For this review, take the finished solid that the model builds, in its own axes (mm). A direction names the side the tool comes from. Coordinates: 2 decimals unless noted, no trailing zeros. Order: outer loops, then holes, each group sorted by start corner. A loop starts at its lowest first (then second) coordinate and runs counter-clockwise, first axis right, second up.
from build123d import *

# Parameters (mm, degrees)
SKETCH_1_W                  = 105
SKETCH_1_H                  = 40
EXTRUDE_1_DEPTH             = 18
SKETCH_2_W                  = 30
SKETCH_2_H                  = 40
CUT_EXTRUDE_1_DEPTH         = 5
SKETCH_3_W                  = 60
SKETCH_3_H                  = 40
CUT_EXTRUDE_2_DEPTH         = 6.5
HOLE_WIZARD_1_D             = 6.6
HOLE_WIZARD_1_CBORE_D       = 11
HOLE_WIZARD_1_CBORE_DEPTH   = 6.8
SKETCH_6_R                  = 5
CUT_EXTRUDE_3_DEPTH         = 2
SKETCH_7_R                  = 14
CUT_EXTRUDE_4_DEPTH         = 8
SKETCH_8_R                  = 12.5
CUT_EXTRUDE_5_DEPTH         = 59.021547722
CHAMFER_1_SIZE              = 3
HOLE_WIZARD_M5_1_AT_2_COUNT = 2
HOLE_WIZARD_M5_1_AT_2_PITCH = 10


with BuildPart() as part:
    # 草图1 → 凸台-拉伸1 (new body)
    with BuildSketch(Plane.XY):
        Rectangle(SKETCH_1_W, SKETCH_1_H)
    extrude(amount=EXTRUDE_1_DEPTH)

    # 草图2 → 切除-拉伸1 (cut)
    with BuildSketch(Plane(origin=(0, 0, 0), x_dir=(-1, 0, 0), z_dir=(0, 0, -1))):
        with Locations((37.5, 0)):
            Rectangle(SKETCH_2_W, SKETCH_2_H)
    extrude(amount=-CUT_EXTRUDE_1_DEPTH, mode=Mode.SUBTRACT)

    # 草图3 → 切除-拉伸2 (cut)
    with BuildSketch(Plane(origin=(0, 0, 0), x_dir=(-1, 0, 0), z_dir=(0, 0, -1))):
        with Locations((-22.5, 0)):
            Rectangle(SKETCH_3_W, SKETCH_3_H)
    extrude(amount=-CUT_EXTRUDE_2_DEPTH, mode=Mode.SUBTRACT)

    # 打孔尺寸(%根据)内六角圆柱头螺钉的类型1 (through all)
    with Locations(Plane.XY.offset(18)):
        with Locations((-46, 0), (-30.5, 0), (-15, 0)):
            CounterBoreHole(HOLE_WIZARD_1_D / 2, HOLE_WIZARD_1_CBORE_D / 2, HOLE_WIZARD_1_CBORE_DEPTH)

    # 草图6 → 切除-拉伸3 (cut)
    with BuildSketch(Plane(origin=(0, 0, 0), x_dir=(-1, 0, 0), z_dir=(0, 0, -1))):
        with Locations((15, 0)):
            Circle(SKETCH_6_R)
    extrude(amount=-CUT_EXTRUDE_3_DEPTH, mode=Mode.SUBTRACT)

    # 草图7 → 切除-拉伸4 (cut)
    with BuildSketch(Plane(origin=(0, 0, 6.5), x_dir=(-1, 0, 0), z_dir=(0, 0, -1))):
        with Locations((-17.5, 0)):
            Circle(SKETCH_7_R)
    extrude(amount=-CUT_EXTRUDE_4_DEPTH, mode=Mode.SUBTRACT)

    # 草图8 → 切除-拉伸5 (cut, through all)
    with BuildSketch(Plane(origin=(0, 0, 14.5), x_dir=(-1, 0, 0), z_dir=(0, 0, -1))):
        with Locations((-17.5, 0)):
            Circle(SKETCH_8_R)
    extrude(amount=-CUT_EXTRUDE_5_DEPTH, mode=Mode.SUBTRACT)

    # 倒角1
    chamfer_1_edges = [part.edges().sort_by_distance(p)[0] for p in [
        (-22.5, -20, 2.5),
        (-22.5, 20, 2.5),
        (-7.5, 20, 3.25),
        (-7.5, -20, 3.25),
        (52.5, -20, 12.25),
        (-52.5, -20, 11.5),
        (-52.5, 20, 11.5),
        (52.5, 20, 12.25),
    ]]
    chamfer(chamfer_1_edges, length=CHAMFER_1_SIZE)

    # 草图10 → M5 螺纹孔1 (revolve, cut)
    with BuildSketch(Plane(origin=(44.5, -20, 12.5), x_dir=(0, 0, -1), z_dir=(1, 0, 0))):
        Polygon((0, 0), (0, 13.6618073), (2.1, 12.4), (2.1, 0), align=None)
    hole_wizard_m5_1 = revolve(axis=Axis((44.5, -26.35, 12.5), (0, 1, 0)), mode=Mode.SUBTRACT)

    # M5 螺纹孔1 at 2: M5 螺纹孔1 ×2
    with Locations(*[(-i * HOLE_WIZARD_M5_1_AT_2_PITCH, 0, 0) for i in range(1, HOLE_WIZARD_M5_1_AT_2_COUNT)]):
        add(hole_wizard_m5_1, mode=Mode.SUBTRACT)

    # 镜向1: M5 螺纹孔1 across plane
    add(hole_wizard_m5_1.mirror(Plane.ZX), mode=Mode.SUBTRACT)

    # 镜向1 copy 1 sketch → 镜向1 copy 1 (revolve, cut)
    with BuildSketch(Plane(origin=(34.5, 20, 12.5), x_dir=(0, 0, -1), z_dir=(1, 0, 0))):
        Polygon((0, 0), (0, -13.6618073), (2.1, -12.4), (2.1, 0), align=None)
    revolve(axis=Axis((34.5, 26.35, 12.5), (0, 1, 0)), mode=Mode.SUBTRACT)


solid = part.part
1. Machinability: for faces 5 (the face through (-21, 18.5, 2.5)), 6 (the face through (-7.5, 0, 3)), 7 (the face through (44.39, -6.56, 12.15)), 8 (the face through (-36, 0, 15)), 9 (the face through (22.8, 11.5, 14.5)), which of the approach directions +Z, -Z, +X, -X, +Y, -Y give a long, thin tool a straight path to every point of the face, cutting with its end or side? Answer none if there is none.
Answer below:
face 5: -Z, -X, +Y
face 6: -Z, +X, +Y, -Y
face 7: -Y
face 8: +Z
face 9: -Z
2. The part is to be moulded in two halves that separate along Y. For faces 1 (the face through (51, 18.5, 12.2)), 2 (the face through (-51.495, 0.242, 14.648)), 3 (the face through (-15, -4, 11.2)), 4 (the face through (52.5, 0, 12)), say which applies: +Y half, -Y half, draft (parallel to the pull), parting line (faces both ways), or undercut.
Answer below:
face 1: +Y half
face 2: undercut
face 3: undercut
face 4: draft
3. Take a section at D-D, the plane y = 16. Give the boundary of the cut face in (x, z).
Answer below:
outline: (-52.5, 5) - (-22.5, 5) - (-22.5, 0) - (-7.5, 0) - (-7.5, 6.5) - (52.5, 6.5) - (52.5, 18) - (-52.5, 18) - close; hole circle Ø4.2 at (34.5, 12.5); hole circle Ø4.2 at (44.5, 12.5)
4. Take a section at C-C, the plane y = -10.5. Give the boundary of the cut face in (x, z).
Answer below:
outline: (-52.5, 5) - (-22.5, 5) - (-22.5, 0) - (-7.5, 0) - (-7.5, 6.5) - (8.24, 6.5) - (8.24, 14.5) - (10.72, 14.5) - (10.72, 18) - (-52.5, 18) - close; (24.28, 14.5) - (26.76, 14.5) - (26.76, 6.5) - (52.5, 6.5) - (52.5, 18) - (24.28, 18) - close; hole circle Ø4.2 at (34.5, 12.5); hole circle Ø4.2 at (44.5, 12.5)
5. Take a section at B-B, the plane z = 8. Give the boundary of the cut face in (x, y), plus the area to 3 significant figures.
Answer below:
outline: (-52.5, -17) - (-49.5, -20) - (49.5, -20) - (52.5, -17) - (52.5, 17) - (49.5, 20) - (-49.5, 20) - (-52.5, 17) - close; hole circle Ø6.6 at (-46, 0); hole circle Ø6.6 at (-30.5, 0); hole circle Ø6.6 at (-15, 0); hole circle Ø28 at (17.5, 0)
area: 3,460 mm2
6. Clearance check with flat-ended pins moving along their axes: pin 1 Ø3.5 at (x, y) = (-17, 2.5) entering from +Z; pin 2 Ø5.5 at (x, y) = (-30.5, 0) entering from -Z; pin 3 Ø2.5 at (y, z) = (-4, 3) entering from -X; pin 4 Ø3.5 at (x, z) = (44.5, 12.5) entering from +Y. State where each tip first meets the part, or that it passes through.
Answer below:
pin 1: stops at z = 11.2
pin 2: passes through
pin 3: stops at x = -22.5
pin 4: stops at y = 7.39
7. To check wall thickness, follow L1, parallel to X at y = -12, z = 12.5; L2, parallel to X at y = 15.5, z = 12.5; L3, parallel to X at y = 13, z = 14.25. State the ranges of each line that lie inside material, in increasing order.
Answer below:
L1: x = -52.5 to 10.29, 24.71 to 32.4, 36.6 to 42.4, 46.6 to 52.5
L2: x = -52.5 to 32.4, 36.6 to 42.4, 46.6 to 52.5
L3: x = -52.5 to 12.3, 22.7 to 33.34, 35.66 to 43.34, 45.66 to 52.5
8. Take a section at A-A, the plane x = -46. Give the boundary of the cut face in (y, z).
Answer below:
outline: (-20, 5) - (-3.3, 5) - (-3.3, 11.2) - (-5.5, 11.2) - (-5.5, 18) - (-20, 18) - close; (3.3, 5) - (20, 5) - (20, 18) - (5.5, 18) - (5.5, 11.2) - (3.3, 11.2) - close
